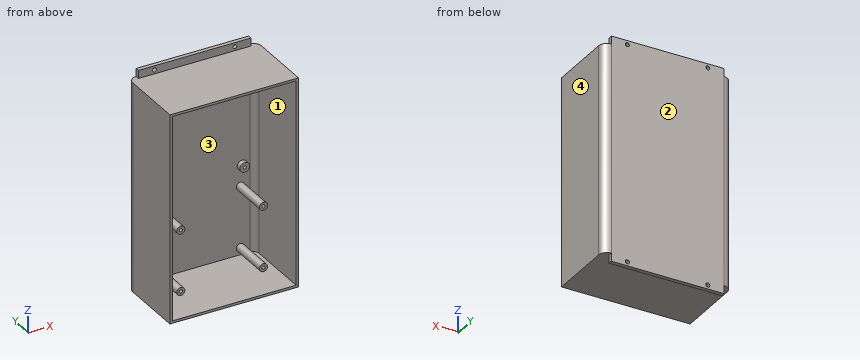
from build123d import *

# Parameters (mm, degrees)
SKETCH1_W           = 160
SKETCH1_H           = 90
BOSS_EXTRUDE1_DEPTH = 260
FILLET2_R           = 10
SHELL1_T            = -3
SKETCH2_R           = 5
SKETCH2_R_2         = 2
BOSS_EXTRUDE2_DEPTH = 50
SKETCH3_R           = 6
SKETCH3_R_2         = 2
BOSS_EXTRUDE3_DEPTH = 6
SKETCH4_W           = 140
SKETCH4_H           = 5
BOSS_EXTRUDE4_DEPTH = 10
SKETCH5_W           = 140
SKETCH5_H           = 5
BOSS_EXTRUDE5_DEPTH = 10
SKETCH6_R           = 2.5
CUT_EXTRUDE1_DEPTH  = 326.153809758


with BuildPart() as part:
    # Sketch1 → Boss-Extrude1 (new body)
    with BuildSketch(Plane.XY):
        with Locations((80, 45)):
            Rectangle(SKETCH1_W, SKETCH1_H)
    extrude(amount=BOSS_EXTRUDE1_DEPTH)

    # Fillet2
    fillet2_edges = [part.edges().sort_by_distance(p)[0] for p in [
        (0, 90, 130),
        (160, 90, 130),
    ]]
    fillet(fillet2_edges, radius=FILLET2_R)

    # Shell1
    shell1_openings = [part.faces().sort_by_distance(p)[0] for p in [
        (80, 0, 130),
    ]]
    offset(amount=SHELL1_T, openings=shell1_openings, kind=Kind.INTERSECTION)

    # Sketch2 → Boss-Extrude2 (add)
    # profile 1 of 4: a face of its own
    with BuildSketch(Plane(origin=(0, 87, 0), x_dir=(-1, 0, 0), z_dir=(0, -1, 0))):
        with Locations(Location((-35, -88.2, 0), (0, 0, 90))):
            Circle(SKETCH2_R)
        with Locations(Location((-35, -88.2, 0), (0, 0, 90))):
            Circle(SKETCH2_R_2, mode=Mode.SUBTRACT)
    # profile 2 of 4: a face of its own
    with BuildSketch(Plane(origin=(0, 87, 0), x_dir=(-1, 0, 0), z_dir=(0, -1, 0))):
        with Locations(Location((-35, -12, 0), (0, 0, 90))):
            Circle(SKETCH2_R)
        with Locations(Location((-35, -12, 0), (0, 0, 90))):
            Circle(SKETCH2_R_2, mode=Mode.SUBTRACT)
    # profile 3 of 4: a face of its own
    with BuildSketch(Plane(origin=(0, 87, 0), x_dir=(-1, 0, 0), z_dir=(0, -1, 0))):
        with Locations(Location((-137.87, -12, 0), (0, 0, 90))):
            Circle(SKETCH2_R)
        with Locations(Location((-137.87, -12, 0), (0, 0, 90))):
            Circle(SKETCH2_R_2, mode=Mode.SUBTRACT)
    # profile 4 of 4: a face of its own
    with BuildSketch(Plane(origin=(0, 87, 0), x_dir=(-1, 0, 0), z_dir=(0, -1, 0))):
        with Locations(Location((-137.87, -88.2, 0), (0, 0, 90))):
            Circle(SKETCH2_R)
        with Locations(Location((-137.87, -88.2, 0), (0, 0, 90))):
            Circle(SKETCH2_R_2, mode=Mode.SUBTRACT)
    extrude(amount=BOSS_EXTRUDE2_DEPTH)

    # Sketch3 → Boss-Extrude3 (add)
    # profile 1 of 4: a face of its own
    with BuildSketch(Plane(origin=(0, 87, 0), x_dir=(-1, 0, 0), z_dir=(0, -1, 0))):
        with Locations(Location((-20, -114, 0), (0, 0, 90))):
            Circle(SKETCH3_R)
        with Locations(Location((-20, -114, 0), (0, 0, 90))):
            Circle(SKETCH3_R_2, mode=Mode.SUBTRACT)
    # profile 2 of 4: a face of its own
    with BuildSketch(Plane(origin=(0, 87, 0), x_dir=(-1, 0, 0), z_dir=(0, -1, 0))):
        with Locations(Location((-20, -250, 0), (0, 0, 90))):
            Circle(SKETCH3_R)
        with Locations(Location((-20, -250, 0), (0, 0, 90))):
            Circle(SKETCH3_R_2, mode=Mode.SUBTRACT)
    # profile 3 of 4: a face of its own
    with BuildSketch(Plane(origin=(0, 87, 0), x_dir=(-1, 0, 0), z_dir=(0, -1, 0))):
        with Locations(Location((-140, -114, 0), (0, 0, 90))):
            Circle(SKETCH3_R)
        with Locations(Location((-140, -114, 0), (0, 0, 90))):
            Circle(SKETCH3_R_2, mode=Mode.SUBTRACT)
    # profile 4 of 4: a face of its own
    with BuildSketch(Plane(origin=(0, 87, 0), x_dir=(-1, 0, 0), z_dir=(0, -1, 0))):
        with Locations(Location((-140, -250, 0), (0, 0, 90))):
            Circle(SKETCH3_R)
        with Locations(Location((-140, -250, 0), (0, 0, 90))):
            Circle(SKETCH3_R_2, mode=Mode.SUBTRACT)
    extrude(amount=BOSS_EXTRUDE3_DEPTH)

    # Sketch4 → Boss-Extrude4 (add)
    with BuildSketch(Plane(origin=(0, 0, 0), x_dir=(-1, 0, 0), z_dir=(0, 0, -1))):
        with Locations((-80, 87.5)):
            Rectangle(SKETCH4_W, SKETCH4_H)
    extrude(amount=BOSS_EXTRUDE4_DEPTH)

    # Sketch5 → Boss-Extrude5 (add)
    with BuildSketch(Plane.XY.offset(260)):
        with Locations((80, 87.5)):
            Rectangle(SKETCH5_W, SKETCH5_H)
    extrude(amount=BOSS_EXTRUDE5_DEPTH)

    # Sketch6 → Cut-Extrude1 (cut, through all)
    with BuildSketch(Plane(origin=(0, 85, 0), x_dir=(-1, 0, 0), z_dir=(0, -1, 0))):
        with Locations(Location((-130, -265, 0), (0, 0, 180))):
            Circle(SKETCH6_R)
        with Locations(Location((-30, -265, 0), (0, 0, 180))):
            Circle(SKETCH6_R)
        with Locations(Location((-130, 5, 0), (0, 0, 180))):
            Circle(SKETCH6_R)
        with Locations(Location((-30, 5, 0), (0, 0, 180))):
            Circle(SKETCH6_R)
    extrude(amount=-CUT_EXTRUDE1_DEPTH, mode=Mode.SUBTRACT)


solid = part.part
CAD build for the part. Positions are in the model's coordinates, mm. Face numbers are marked on the shaded views. A direction names the side the tool comes from. Round coordinates to 2 decimals unless told otherwise and drop trailing zeros. Write each loop counter-clockwise with the first axis right and the second up, starting at its lowest first coordinate (ties: lowest second). Pieces come first, ordered by that corner, then holes. Notation, with made-up numbers: M -20,80 L -7,80 A17 ccw -7,87 Z; hole C 58.5,60 d3. An arc over 180 degrees is marked long. Use a Markdown table: item, result. Add a question column.
1. Slice it at D-D on z = 150.5. Give the cut face in (x, y).
2. Slice it at B-B on y = 16. Give the cut face in (x, z), then the cut area to 3 significant figures.
3. Drill centre lines: probe 1 along Z at (x, y) = (130, 88.1); probe 2 along Z at (x, y) = (111.5, 44); probe 3 along X at (y, z) = (53, 179). Where is each one in solid material? Low to high.
4. Slice it at A-A on y = 56. Give the number of separate pieces and of enclosed holes in the cut face, then the cut area to 3 significant figures.
5. Slice it at C-C on x = 81.5. Give the cut face in (y, z), then the cut area to 3 significant figures.
6. 3-axis set-ups, long thin cutter, end or side, ignore diameter. For the marked faces 1 and 2: which of +Z, -Z, +X, -X, +Y, -Y reach the whole face in a straight line?
7. Flat gauge pins, fed straight in: P1, Ø9.5, axis at x = 140, z = 111.5, coming from the -Y side; P2, Ø4.5, axis at x = 138.5, z = 88.5, coming from the -Y side; P3, Ø1.5, axis at y = 88, z = 263, coming from the +X side; P4, Ø3, axis at x = 30, z = -5, coming from the -Y side. Where does each tip first touch, or does it go through?
8. Pull direction Z, two halves, no side cores. Call the marked faces 3 and 4: released by +Z, released by -Z, zero draft, split by the parting line, or undercut.
Reply:
| question | item | result |
|---|---|---|
| 1 | outline | M 0,0 L 3,0 L 3,80 A7 cw 10,87 L 150,87 A7 cw 157,80 L 157,0 L 160,0 L 160,80 A10 ccw 150,90 L 10,90 A10 ccw 0,80 Z |
| 2 | outline | M 0,0 L 160,0 L 160,260 L 0,260 Z; hole M 3,3 L 157,3 L 157,257 L 3,257 Z |
| 2 | area | 2,480 mm^2 |
| 3 | probe 1 | z = -10 to -7.5, -2.5 to 262.5, 267.5 to 270 |
| 3 | probe 2 | z = 0 to 3, 257 to 260 |
| 3 | probe 3 | x = 0 to 3, 157 to 160 |
| 4 | separate pieces | 5 |
| 4 | enclosed holes | 5 |
| 4 | area | 2,750 mm^2 |
| 5 | outline | M 0,0 L 85,0 L 85,-10 L 90,-10 L 90,270 L 85,270 L 85,260 L 0,260 L 0,257 L 87,257 L 87,3 L 0,3 Z |
| 5 | area | 1,400 mm^2 |
| 6 | face 1 | -Y |
| 6 | face 2 | +Z, -Z, +X, -X, +Y |
| 7 | P1 | stops at y = 81 |
| 7 | P2 | stops at y = 37 |
| 7 | P3 | stops at x = 150 |
| 7 | P4 | passes through |
| 8 | face 3 | undercut |
| 8 | face 4 | zero draft |
